The listing builds one solid part. Answer for the finished solid, in the listing's coordinates (mm). Face numbers are marked on the shaded views. A direction names the side the tool comes from. Give positions to 0.01 mm unless a question says otherwise; leave off trailing zeros. Loops run counter-clockwise (first coordinate to the right, second up) from the corner with the lowest first, then second, coordinate; pieces in that order, holes last. Notation, with made-up numbers: (6, 32) -> (19, 32) arc R16 cw to (19, 58) -> close; hole circle Ø7 at (29.25, -31.75). An arc over 180 degrees is marked (long way). One line per question, with ' | ' between items. Start each with the question number.
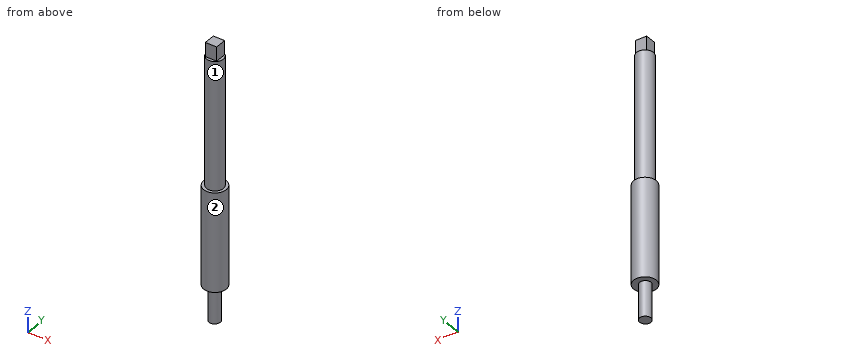
from build123d import *

# Parameters (mm, degrees)
SKETCH_1_R      = 5.95
EXTRUDE_1_DEPTH = 91
SKETCH_2_W      = 8
SKETCH_2_H      = 8
EXTRUDE_2_DEPTH = 10
SKETCH_3_R      = 8
EXTRUDE_3_DEPTH = 70
SKETCH_4_R      = 4
EXTRUDE_4_DEPTH = 25


with BuildPart() as part:
    # 草图1 → 凸台-拉伸1 (new body)
    with BuildSketch(Plane.XY):
        Circle(SKETCH_1_R)
    extrude(amount=EXTRUDE_1_DEPTH)

    # 草图2 → 凸台-拉伸2 (add)
    with BuildSketch(Plane.XY.offset(91)):
        Rectangle(SKETCH_2_W, SKETCH_2_H)
    extrude(amount=EXTRUDE_2_DEPTH)

    # 草图3 → 凸台-拉伸3 (add)
    with BuildSketch(Plane(origin=(0, 0, 0), x_dir=(-1, 0, 0), z_dir=(0, 0, -1))):
        Circle(SKETCH_3_R)
    extrude(amount=EXTRUDE_3_DEPTH)

    # 草图4 → 凸台-拉伸4 (add)
    with BuildSketch(Plane(origin=(0, 0, -70), x_dir=(-1, 0, 0), z_dir=(0, 0, -1))):
        with Locations((0.224619263, 0)):
            Circle(SKETCH_4_R)
    extrude(amount=EXTRUDE_4_DEPTH)


solid = part.part
1. Straight lines are drawn through the part: L1, parallel to X at y = -0.5, z = -44.5; L2, parallel to Z at x = 3.75, y = 1; L3, parallel to Z at x = -2.75, y = -4.25. For each, find the intervals that lie inside material, in ascending order.
2. The part is cut by section C-C (z = 62). Write down the section's boundary in (x, y), plus the area to 3 significant figures.
3. Each of these flat-tipped pins is pushed along its axis until it touches: pin 1 Ø3 at (y, z) = (-5.5, 69) entering from +X; pin 2 Ø9 at (x, z) = (-1, 94.5) entering from +Y; pin 3 Ø5 at (x, y) = (-6.5, -6) entering from -Z. Where does it stop, or does it pass through?
4. The part is cut by section D-D (z = -62.5). Write down the section's boundary in (x, y).
5. For the marked faces 1 and 2, determine the directions among +Z, -Z, +X, -X, +Y, -Y from which every point of the face is accessible in a straight line to the end or side of a thin tool.
6. The part is cut by section A-A (y = 0). Write down the section's boundary in (x, z), plus the area to 3 significant figures.
7. The part is cut by section B-B (x = 0). Write down the section's boundary in (y, z), plus the area to 3 significant figures.
Check sheet entries:
1) L1: x = -7.98 to 7.98 | L2: z = -70 to 101 | L3: z = -70 to 91
2) outline: circle Ø11.9 at (0, 0) | area: 111 mm^2
3) pin 1: stops at x = 4.4 | pin 2: stops at y = 5.95 | pin 3: stops at z = -70
4) outline: circle Ø16 at (0, 0)
5) face 1: +Z | face 2: +Z, -Z
6) outline: (-8, -70) -> (-4.22, -70) -> (-4.22, -95) -> (3.78, -95) -> (3.78, -70) -> (8, -70) -> (8, 0) -> (5.95, 0) -> (5.95, 91) -> (4, 91) -> (4, 101) -> (-4, 101) -> (-4, 91) -> (-5.95, 91) -> (-5.95, 0) -> (-8, 0) -> close | area: 2,480 mm^2
7) outline: (-8, -70) -> (-3.99, -70) -> (-3.99, -95) -> (3.99, -95) -> (3.99, -70) -> (8, -70) -> (8, 0) -> (5.95, 0) -> (5.95, 91) -> (4, 91) -> (4, 101) -> (-4, 101) -> (-4, 91) -> (-5.95, 91) -> (-5.95, 0) -> (-8, 0) -> close | area: 2,480 mm^2
